```python
from build123d import *

# Parameters (mm, degrees)
BOSS_EXTRUDE1_DEPTH      = 40
BOSS_EXTRUDE1_DEPTH_BACK = 40
SKETCH1_R                = 50
CUT_EXTRUDE1_START       = -20
SKETCH2_R                = 75
SKETCH2_R_2              = 50
CUT_EXTRUDE1_DEPTH       = 20
CUT_EXTRUDE2_START       = -20
CUT_EXTRUDE2_DEPTH       = 20
BOSS_EXTRUDE2_DEPTH      = 20
BOSS_EXTRUDE2_DEPTH_BACK = 100
SKETCH4_W                = 430
SKETCH4_H                = 18
SKETCH5_R                = 15
BOSS_EXTRUDE3_DEPTH      = 4
BOSS_EXTRUDE4_DEPTH      = 10


with BuildPart() as part:
    # Sketch1 → Boss-Extrude1 (new, two sides: drawn at the far end of the back side and taken through both)
    with BuildSketch(Plane(origin=(0, 0, 0), x_dir=(1, 0, 0), z_dir=(0, 1, 0)).offset(-BOSS_EXTRUDE1_DEPTH_BACK)):
        with BuildLine():
            Line((-175, -170), (175, -170))
            Line((175, -170), (82.10152682, 36.869218785))
            ThreePointArc((82.10152682, 36.869218785), (0, 90), (-82.10152682, 36.869218785))
            Line((-82.10152682, 36.869218785), (-175, -170))
        make_face()
        with Locations(Location((0, 0, 0), (0, 0, 270))):
            Circle(SKETCH1_R, mode=Mode.SUBTRACT)
    extrude(amount=BOSS_EXTRUDE1_DEPTH + BOSS_EXTRUDE1_DEPTH_BACK)

    # Sketch2 → Cut-Extrude1 (cut)
    with BuildSketch(Plane(origin=(0, 40, 0), x_dir=(1, 0, 0), z_dir=(0, 1, 0)).offset(CUT_EXTRUDE1_START)):
        with Locations(Location((0, 0, 0), (0, 0, 270))):
            Circle(SKETCH2_R)
        with Locations(Location((0, 0, 0), (0, 0, 270))):
            Circle(SKETCH2_R_2, mode=Mode.SUBTRACT)
    extrude(amount=CUT_EXTRUDE1_DEPTH, mode=Mode.SUBTRACT)

    # Sketch3 → Cut-Extrude2 (cut)
    with BuildSketch(Plane(origin=(0, 40, 0), x_dir=(1, 0, 0), z_dir=(0, 1, 0)).offset(CUT_EXTRUDE2_START)):
        with BuildLine():
            Line((-87.802752727, -19.765541064), (-147.18509781, -152))
            Line((-147.18509781, -152), (147.18509781, -152))
            Line((147.18509781, -152), (87.802752727, -19.765541064))
            ThreePointArc((87.802752727, -19.765541064), (0, -90), (-87.802752727, -19.765541064))
        make_face()
    cut_extrude2 = extrude(amount=CUT_EXTRUDE2_DEPTH, mode=Mode.SUBTRACT)

    # Mirror1: Cut-Extrude2 across plane
    add(cut_extrude2.mirror(Plane.ZX), mode=Mode.SUBTRACT)

    # Sketch4 → Boss-Extrude2 (add, two sides: drawn at the far end of the back side and taken through both)
    with BuildSketch(Plane(origin=(0, 40, 0), x_dir=(1, 0, 0), z_dir=(0, 1, 0)).offset(-BOSS_EXTRUDE2_DEPTH_BACK)):
        with Locations((0, -161)):
            Rectangle(SKETCH4_W, SKETCH4_H)
    extrude(amount=BOSS_EXTRUDE2_DEPTH + BOSS_EXTRUDE2_DEPTH_BACK)

    # Sketch5 → Boss-Extrude3 (add)
    with BuildSketch(Plane(origin=(0, 0, 152), x_dir=(-1, 0, 0), z_dir=(0, 0, -1))):
        with Locations(Location((-190, 35, 0), (0, 0, 180))):
            Circle(SKETCH5_R)
        with Locations(Location((-190, -35, 0), (0, 0, 180))):
            Circle(SKETCH5_R)
        with Locations(Location((190, -35, 0), (0, 0, 180))):
            Circle(SKETCH5_R)
        with Locations(Location((190, 35, 0), (0, 0, 180))):
            Circle(SKETCH5_R)
    extrude(amount=BOSS_EXTRUDE3_DEPTH)

    # Sketch6 → Boss-Extrude4 (add)
    with BuildSketch(Plane(origin=(0, 0, 148), x_dir=(-1, 0, 0), z_dir=(0, 0, -1))):
        Polygon((-179.344928978, 35), (-184.672464489, 44.227562184), (-195.327535511, 44.227562184), (-200.655071022, 35), (-195.327535511, 25.772437816), (-184.672464489, 25.772437816), align=None)
        Polygon((-179.344928978, -38.24088904), (-181.86577225, -27.392882336), (-192.520843272, -24.151993296), (-200.655071022, -31.75911096), (-198.13422775, -42.607117664), (-187.479156728, -45.848006704), align=None)
        Polygon((199.191466328, 30.386218908), (198.591384797, 40.653152792), (189.399918469, 45.266933884), (180.808533672, 39.613781092), (181.408615203, 29.346847208), (190.600081531, 24.733066116), align=None)
        Polygon((199.191466328, -38.24088904), (197.402425403, -28.660401182), (188.210959075, -25.419512142), (180.808533672, -31.75911096), (182.597574597, -41.339598818), (191.789040925, -44.580487858), align=None)
    extrude(amount=BOSS_EXTRUDE4_DEPTH)


solid = part.part
```
Can you work these out from the model? Positions are in its coordinate system, mm. A direction names the side the tool comes from. Coordinates: 2 decimals unless noted, no trailing zeros. Loops run counter-clockwise (first coordinate to the right, second up) from the corner with the lowest first, then second, coordinate; pieces in that order, holes last. Notation, with made-up numbers: (71.5, 78.5) - (105.5, 78.5) arc R22 ccw to (105.5, 102.5) - close; hole circle Ø9 at (-26, -9). An arc over 180 degrees is marked (long way). Use a Markdown table: item, result.
Item 1: For faces 4 (the face through (117.91, 29.86, 86.81)), 5 (the face through (192.9, -44.2, 143.1)), 6 (the face through (117.91, -29.86, 86.81)), 7 (the face through (181.97, 39.55, 143.07)), which set-ups out of +Z, -Z, +X, -X, +Y, -Y let a thin tool reach every point of the face, with its end or its side?
Numbers:
| item | result |
|---|---|
| face 4 | +Y |
| face 5 | -Z, +X, -Y |
| face 6 | -Y |
| face 7 | -Z, +Y |
Item 2: I want a section at C-C on y = 1.5. Please give me the cut outline in (x, z), and give its area (3 significant figures).
Numbers:
| item | result |
|---|---|
| outline | (-215, 152) - (-166.92, 152) - (-82.1, -36.87) arc R90 ccw to (82.1, -36.87) - (166.92, 152) - (215, 152) - (215, 170) - (-215, 170) - close; hole circle Ø100 at (0, 0) |
| area | 53,200 mm2 |
Item 3: Will these pins go through, and if not, where does the flat tip stop? pin 1 (9 mm diameter, centred on x = 189.5, y = -29, fed in from -Z); pin 2 (6 mm diameter, centred on x = -114.5, z = 95, fed in from -Y); pin 3 (1.5 mm diameter, centred on x = 106, y = 32.5, fed in from -Z); pin 4 (12 mm diameter, centred on x = 31, z = 22, fed in from +Y).
Numbers:
| item | result |
|---|---|
| pin 1 | stops at z = 138 |
| pin 2 | stops at y = -20 |
| pin 3 | stops at z = 14.68 |
| pin 4 | passes through |
Item 4: I want a section at B-B on z = 0. Please give me the cut outline in (x, y).
Numbers:
| item | result |
|---|---|
| outline | (-98.66, -40) - (-50, -40) - (-50, 20) - (-75, 20) - (-75, 40) - (-98.66, 40) - close; (50, -40) - (98.66, -40) - (98.66, 40) - (75, 40) - (75, 20) - (50, 20) - close |
Item 5: I want a section at D-D on x = 68. Please give me the cut outline in (y, z), and give its area (3 significant figures).
Numbers:
| item | result |
|---|---|
| outline | (-60, 152) - (-20, 152) - (-20, 58.96) - (-40, 58.96) - (-40, -58.96) - (40, -58.96) - (40, -31.64) - (20, -31.64) - (20, 31.64) - (40, 31.64) - (40, 58.96) - (20, 58.96) - (20, 152) - (60, 152) - (60, 170) - (-60, 170) - close |
| area | 14,000 mm2 |
Item 6: I want a section at A-A on x = 0. Please give me the cut outline in (y, z), and give its area (3 significant figures).
Numbers:
| item | result |
|---|---|
| outline | (-60, 152) - (-20, 152) - (-20, 90) - (-40, 90) - (-40, 50) - (20, 50) - (20, 75) - (40, 75) - (40, 90) - (20, 90) - (20, 152) - (60, 152) - (60, 170) - (-60, 170) - close; (-40, -90) - (40, -90) - (40, -75) - (20, -75) - (20, -50) - (-40, -50) - close |
| area | 10,000 mm2 |
Item 7: If I drill on probe 1 along Y at (x, z) = (152.5, 139.5); probe 2 along Y at (x, z) = (16, 148); probe 3 along X at (y, z) = (27, 31), over which ranges is the centre line in solid material (lowest first)? Write a range as from..to.
Numbers:
| item | result |
|---|---|
| probe 1 | y = -40..40 |
| probe 2 | y = -20..20 |
| probe 3 | x = -112.58..-92.85, -84.49..-68.29, 68.29..84.49, 92.85..112.58 |
Item 8: We'd pull the mould along X, two halves only. Please class faces 1 (the face through (196.53, -27.9, 143.07)), 2 (the face through (1.45, -0.56, -89.99)), 3 (the face through (180.59, -32.89, 143.07)): released by +X, released by -X, zero draft, split by the parting line, or undercut.
Numbers:
| item | result |
|---|---|
| face 1 | released by +X |
| face 2 | split by the parting line |
| face 3 | undercut |
